Here's how the part is built. I have some questions about the finished solid (model axes, mm). Round coordinates to 2 decimals unless told otherwise and drop trailing zeros. Loops run counter-clockwise (first coordinate to the right, second up) from the corner with the lowest first, then second, coordinate; pieces in that order, holes last. Notation, with made-up numbers: M 88,19 L 140,19 A16 cw 140,30 Z; hole C -37.5,71 d7. An arc over 180 degrees is marked long. Answer as a JSON object with one key per item and string values.
from build123d import *

# Parameters (mm, degrees)
SKETCH_1_W          = 130
SKETCH_1_H          = 40
EXTRUDE_1_DEPTH     = 3
SKETCH_2_R          = 7
SKETCH_2_R_2        = 2.15
CUT_EXTRUDE_1_DEPTH = 3
FILLET_1_R          = 5


with BuildPart() as part:
    # 草图1 → 凸台-拉伸1 (new body)
    with BuildSketch(Plane.XY):
        Rectangle(SKETCH_1_W, SKETCH_1_H)
    extrude(amount=EXTRUDE_1_DEPTH)

    # 草图2 → 切除-拉伸1 (cut)
    with BuildSketch(Plane.XY.offset(3)):
        with Locations((-50, 0)):
            Circle(SKETCH_2_R)
        with Locations((50, 0)):
            Circle(SKETCH_2_R)
        with Locations((-6, 6)):
            Circle(SKETCH_2_R_2)
        with Locations((6, 6)):
            Circle(SKETCH_2_R_2)
        with Locations((6, -6)):
            Circle(SKETCH_2_R_2)
        with Locations((-6, -6)):
            Circle(SKETCH_2_R_2)
    extrude(amount=-CUT_EXTRUDE_1_DEPTH, mode=Mode.SUBTRACT)

    # 圆角1
    fillet_1_edges = [part.edges().sort_by_distance(p)[0] for p in [
        (65, -20, 1.5),
        (-65, -20, 1.5),
        (-65, 20, 1.5),
        (65, 20, 1.5),
    ]]
    fillet(fillet_1_edges, radius=FILLET_1_R)


solid = part.part
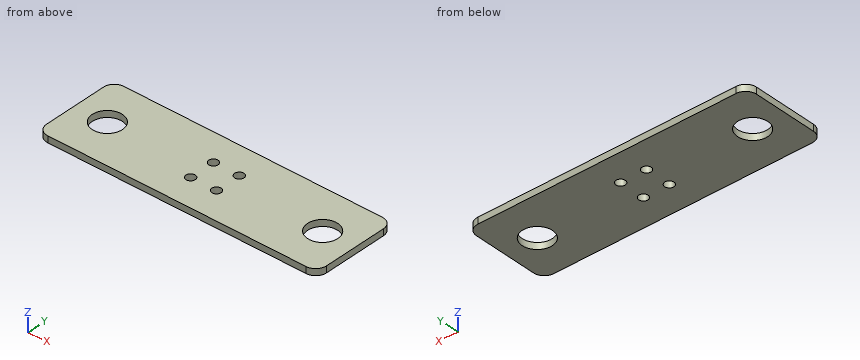
Item 1: I want a section at B-B on z = 0.75. List the corners of the cut face in (x, y) for me, plus the area to 3 significant figures.
Solution:
{"outline": "M -65,-15 A5 ccw -60,-20 L 60,-20 A5 ccw 65,-15 L 65,15 A5 ccw 60,20 L -60,20 A5 ccw -65,15 Z; hole C -50,0 d14; hole C -6,-6 d4.3; hole C -6,6 d4.3; hole C 6,-6 d4.3; hole C 6,6 d4.3; hole C 50,0 d14", "area": "4,810 mm2"}
Item 2: I want a section at D-D on y = -1.5. List the corners of the cut face in (x, z) for me, plus the area to 3 significant figures.
Solution:
{"outline": "M -65,0 L -56.84,0 L -56.84,3 L -65,3 Z; M -43.16,0 L 43.16,0 L 43.16,3 L -43.16,3 Z; M 56.84,0 L 65,0 L 65,3 L 56.84,3 Z", "area": "308 mm2"}
Item 3: I want a section at C-C on x = -50. List the corners of the cut face in (y, z) for me, plus the area to 3 significant figures.
Solution:
{"outline": "M -20,0 L -7,0 L -7,3 L -20,3 Z; M 7,0 L 20,0 L 20,3 L 7,3 Z", "area": "78.0 mm2"}
Item 4: For P1, Ø3.5, axis at x = 6, y = -6, coming from the -Z side, with a flat end and sliding along its axis, tell me the tip position at first contact or that it passes through.
Solution:
{"P1": "passes through"}
Item 5: If I drill on L1, parallel to Y at x = 6, z = 1.7; L2, parallel to X at y = 1.5, z = 2.2; L3, parallel to X at y = -7.5, z = 1, over which ranges is the centre line in solid material (lowest first)? Write a range as from..to.
Solution:
{"L1": "y = -20..-8.15, -3.85..3.85, 8.15..20", "L2": "x = -65..-56.84, -43.16..43.16, 56.84..65", "L3": "x = -65..-7.54, -4.46..4.46, 7.54..65"}
Item 6: I want a section at A-A on x = -6. List the corners of the cut face in (y, z) for me.
Solution:
{"outline": "M -20,0 L -8.15,0 L -8.15,3 L -20,3 Z; M -3.85,0 L 3.85,0 L 3.85,3 L -3.85,3 Z; M 8.15,0 L 20,0 L 20,3 L 8.15,3 Z"}
